Source: CAD feature listing. Evaluate the final solid. Frame: model axes, mm. Face numbers are marked on the shaded views. Give positions to 0.01 mm unless a question says otherwise; leave off trailing zeros. Loops run counter-clockwise (first coordinate to the right, second up) from the corner with the lowest first, then second, coordinate; pieces in that order, holes last.
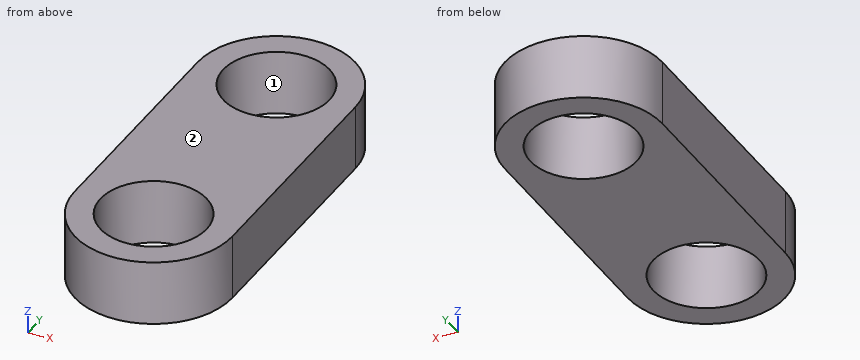
```python
from build123d import *

# Parameters (mm, degrees)
SKETCH1_R           = 3.674588618
BOSS_EXTRUDE1_DEPTH = 4.5


with BuildPart() as part:
    # Sketch1 → Boss-Extrude1 (new body)
    with BuildSketch(Plane.XY):
        with BuildLine():
            Line((31.69623991, -16.220097286), (31.57303389, 0.068183186))
            ThreePointArc((31.57303389, 0.068183186), (26.087023529, 5.47182325), (20.683383464, -0.014187111))
            Line((20.683383464, -0.014187111), (20.806589485, -16.302467582))
            ThreePointArc((20.806589485, -16.302467582), (26.292599845, -21.706107647), (31.69623991, -16.220097286))
        make_face()
        with Locations((26.128208677, 0.026998038)):
            Circle(SKETCH1_R, mode=Mode.SUBTRACT)
        with Locations((26.251414697, -16.261282434)):
            Circle(SKETCH1_R, mode=Mode.SUBTRACT)
    extrude(amount=BOSS_EXTRUDE1_DEPTH)


solid = part.part
```
(1) Section D-D, the plane x = 23.75. Return the cut outline in (y, z), then the cut area to 3 significant figures.
A:
outline: (-21.1, 0) - (-18.95, 0) - (-18.95, 4.5) - (-21.1, 4.5) - close; (-13.57, 0) - (-2.77, 0) - (-2.77, 4.5) - (-13.57, 4.5) - close; (2.83, 0) - (4.93, 0) - (4.93, 4.5) - (2.83, 4.5) - close
area: 67.7 mm2
(2) First-contact query: pin 1 (1.5 mm diameter, centred on y = -19, z = 1.5, fed in from +X). Flat tip, straight axial feed; report the tip coordinate or a pass-through.
A:
pin 1: stops at x = 31.32
(3) Ray query, line 1 along Y through (x, z) = (26.25, 1.5); line 2 along X through (y, z) = (0, 3.3); line 3 along Y through (x, z) = (25.25, 1.1). Return the intervals inside material, ascending.
A:
line 1: y = -21.71 to -19.94, -12.59 to -3.65, 3.7 to 5.47
line 2: x = 20.68 to 22.45, 29.8 to 31.57
line 3: y = -21.61 to -19.8, -12.73 to -3.54, 3.6 to 5.4
(4) Section C-C, the plane z = 1. Return the cut outline in (x, y), then the cut area to 3 significant figures.
A:
outline: (20.68, -0.01) - (20.81, -16.3) arc R5.44 ccw to (31.7, -16.22) - (31.57, 0.07) arc R5.44 ccw to start; hole circle Ø7.35 at (26.13, 0.03); hole circle Ø7.35 at (26.25, -16.26)
area: 186 mm2
(5) Mould query, pull axis Y, two halves, no side actions, for the marked faces 1 and 2. Classes: pulls with the +Y half, pulls with the -Y half, needs draft (parallel to the pull), parting line crosses it, or undercut.
A:
face 1: undercut
face 2: needs draft
(6) Section B-B, the plane y = -18.25. Return the cut outline in (x, z).
A:
outline: (21.18, 0) - (23.16, 0) - (23.16, 4.5) - (21.18, 4.5) - close; (29.34, 0) - (31.32, 0) - (31.32, 4.5) - (29.34, 4.5) - close
(7) Section A-A, the plane x = 27.25. Return the cut outline in (y, z).
A:
outline: (-21.61, 0) - (-19.8, 0) - (-19.8, 4.5) - (-21.61, 4.5) - close; (-12.72, 0) - (-3.47, 0) - (-3.47, 4.5) - (-12.72, 4.5) - close; (3.53, 0) - (5.36, 0) - (5.36, 4.5) - (3.53, 4.5) - close
